from build123d import *

# Parameters (mm, degrees)
BASE_EXTRUDE_DEPTH = 20
FILLET1_R          = 1.2


with BuildPart() as part:
    # Sketch1 → Base-Extrude (new body)
    with BuildSketch(Plane.XY):
        with BuildLine():
            Line((-9, 18), (133, 18))
            Line((133, 18), (133, -18))
            Line((133, -18), (-9, -18))
            ThreePointArc((-9, -18), (-27, 0), (-9, 18))
        make_face()
    extrude(amount=BASE_EXTRUDE_DEPTH)

    # Fillet1
    fillet1_edges = [part.edges().sort_by_distance(p)[0] for p in [
        (-27, 0, 20),
        (62, -18, 20),
        (62, -18, 0),
        (-27, 0, 0),
        (62, 18, 0),
        (62, 18, 20),
    ]]
    fillet(fillet1_edges, radius=FILLET1_R)


solid = part.part
The listing builds one solid part. Answer for the finished solid, in the listing's coordinates (mm). Coordinates: 2 decimals unless noted, no trailing zeros. Order: outer loops, then holes, each group sorted by start corner. A loop starts at its lowest first (then second) coordinate and runs counter-clockwise, first axis right, second up. Notation, with made-up numbers: (2, 7.25) -> (29, 7.25) arc R4 ccw to (29, 13.25) -> close; hole circle Ø5 at (-15, -3.75). An arc over 180 degrees is marked (long way). Answer in a Markdown table with one row per item. Add a question column.
Item 1: Find the intervals of material crossed by L1, parallel to X at y = 6.5, z = 15.75; L2, parallel to X at y = -0.5, z = 6.5; L3, parallel to Y at x = 15.5, z = 19.25, in increasing order. Write a range as from..to.
Item 2: Find section A-A (z = 6.5). Write down the section's boundary in (x, y).
Item 3: This flat-tipped pin is pushed along its axis until it touches: P1, Ø12, axis at y = -13, z = 17, coming from the -X side. Where does it stop, or does it pass through?
Result set:
| question | item | result |
|---|---|---|
| 1 | L1 | x = -25.79..133 |
| 1 | L2 | x = -26.99..133 |
| 1 | L3 | y = -17.91..17.91 |
| 2 | outline | (-9, -18) -> (133, -18) -> (133, 18) -> (-9, 18) arc R18 ccw to start |
| 3 | P1 | stops at x = -25.58 |
